Read the model definition and answer for the solid it produces. Units are mm, in the model's axes. Round coordinates to 2 decimals unless told otherwise and drop trailing zeros. Write each loop counter-clockwise with the first axis right and the second up, starting at its lowest first coordinate (ties: lowest second). Pieces come first, ordered by that corner, then holes. Notation, with made-up numbers: (62, 14) - (100, 14) arc R30 ccw to (100, 42) - close; hole circle Ø7 at (44, -29). An arc over 180 degrees is marked (long way). Use one line per item in the form item = value. Start each with the question number.
1) Consider line 1 along Z through (x, y) = (90, 3.65); line 2 along X through (y, z) = (4.3, -92); line 3 along X through (y, z) = (-2, 103). Determine where each line is inside the solid, lowest interval first. Write a range as from..to.
2) The part is cut by section C-C, the plane x = -90. Give the vertices of the cut face in (y, z).
3) This flat-tipped pin is pushed along its axis until it touches: pin 1 (3.5 mm diameter, centred on x = 88.5, z = 16, fed in from -Y). Where does it stop, or does it pass through?
4) The part is cut by section A-A, the plane z = 18. Give the vertices of the cut face in (x, y), plus the area to 3 significant figures.
5) The part is cut by section B-B, the plane x = 55. Give the vertices of the cut face in (y, z), plus the area to 3 significant figures.
from build123d import *

# Parameters (mm, degrees)
SKETCH_1_W                = 250
SKETCH_1_H                = 306
EXTRUDE_1_DEPTH           = 6
CHAMFER_1_SIZE            = 2
HOLE_WIZARD_M6_1_D        = 5
HOLE_WIZARD_M6_1_DEPTH    = 15
HOLE_WIZARD_M6_1_TIP      = 1.502151548
HOLE_WIZARD_M8_1_D        = 9
HOLE_WIZARD_1_D           = 6.6
HOLE_WIZARD_1_CBORE_D     = 11
HOLE_WIZARD_1_CBORE_DEPTH = 6.8
SKETCH_8_R                = 4
CUT_EXTRUDE_1_DEPTH       = 198.934332545
HOLE_WIZARD_M6_2_D        = 5
CHAMFER_2_SIZE            = 10


with BuildPart() as part:
    # 草图1 → 凸台-拉伸1 (new, symmetric)
    with BuildSketch(Plane(origin=(0, 0, 0), x_dir=(1, 0, 0), z_dir=(0, 1, 0))):
        Rectangle(SKETCH_1_W, SKETCH_1_H)
    extrude(amount=EXTRUDE_1_DEPTH, both=True)

    # 倒角1
    chamfer_1_edges = [part.edges().sort_by_distance(p)[0] for p in [
        (125, 0, 153),
        (-125, 0, 153),
    ]]
    chamfer(chamfer_1_edges, length=CHAMFER_1_SIZE)

    # M6 螺纹孔1
    with Locations(Plane(origin=(0, 0, -153), x_dir=(-1, 0, 0), z_dir=(0, 0, -1))):
        with Locations((-105, 0), (0, 0), (105, 0)):
            Hole(HOLE_WIZARD_M6_1_D / 2, depth=HOLE_WIZARD_M6_1_DEPTH)
            with Locations((0, 0, -(HOLE_WIZARD_M6_1_DEPTH + HOLE_WIZARD_M6_1_TIP / 2))):  # 118° drill point
                Cone(0, HOLE_WIZARD_M6_1_D / 2, HOLE_WIZARD_M6_1_TIP, mode=Mode.SUBTRACT)

    # M8 间隙孔1 (through all)
    with Locations(Plane(origin=(0, 6, 0), x_dir=(1, 0, 0), z_dir=(0, 1, 0))):
        with Locations((-105, -135.00000089), (-55, -135.00000089), (-105, 78.99999911), (-55, 78.99999911), (55, 78.99999911), (105, 78.99999911), (55, -135.00000089), (105, -135.00000089), (-35, -135.00000089), (35, -135.00000089), (-35, 78.99999911), (35, 78.99999911)):
            Hole(HOLE_WIZARD_M8_1_D / 2)

    # 打孔尺寸(%根据)内六角圆柱头螺钉的类型1 (through all)
    with Locations(Plane(origin=(0, -6, 0), x_dir=(-1, 0, 0), z_dir=(0, -1, 0))):
        with Locations((-90, -128), (-90, -18), (-90, 92), (90, 92), (90, -18), (90, -128)):
            CounterBoreHole(HOLE_WIZARD_1_D / 2, HOLE_WIZARD_1_CBORE_D / 2, HOLE_WIZARD_1_CBORE_DEPTH)

    # 草图8 → 切除-拉伸1 (cut, through all)
    with BuildSketch(Plane(origin=(0, 6, 0), x_dir=(1, 0, 0), z_dir=(0, 1, 0))):
        with Locations(Location((0, -135.00000089, 0), (0, 0, 270))):
            Circle(SKETCH_8_R)
        with BuildLine():
            Line((-4, 77.99999911), (-4, 79.99999911))
            ThreePointArc((-4, 79.99999911), (0, 83.99999911), (4, 79.99999911))
            Line((4, 79.99999911), (4, 77.99999911))
            ThreePointArc((4, 77.99999911), (0, 73.99999911), (-4, 77.99999911))
        make_face()
    extrude(amount=-CUT_EXTRUDE_1_DEPTH, mode=Mode.SUBTRACT)

    # M6 螺纹孔2 (through all)
    with Locations(Plane(origin=(0, 6, 0), x_dir=(1, 0, 0), z_dir=(0, 1, 0))):
        with Locations((25, -103), (-25, -103)):
            Hole(HOLE_WIZARD_M6_2_D / 2)

    # 倒角2
    chamfer_2_edges = [part.edges().sort_by_distance(p)[0] for p in [
        (-125, 0, -153),
        (125, 0, -153),
    ]]
    chamfer(chamfer_2_edges, length=CHAMFER_2_SIZE)


solid = part.part
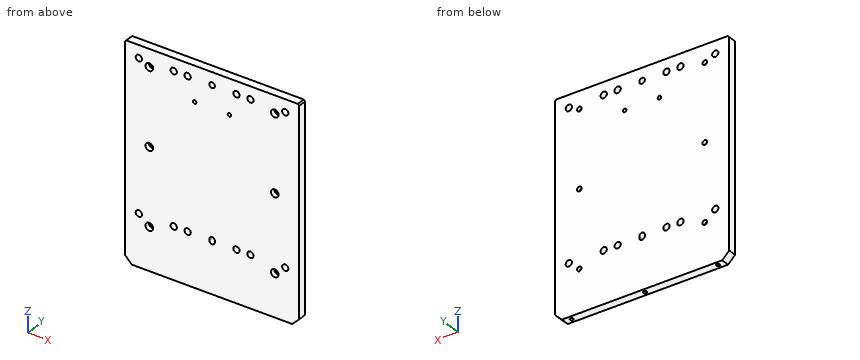
Geometry results:
q1.line_1 = -153..-95.3, -88.7..14.7, 21.3..124.7, 131.3..153
q1.line_2 = -125..-93.3, -86.7..86.7, 93.3..125
q1.line_3 = -125..-27.5, -22.5..22.5, 27.5..125
q2.outline = (-6, -153) - (6, -153) - (6, -95.3) - (0.8, -95.3) - (0.8, -97.5) - (-6, -97.5) - close; (-6, -86.5) - (0.8, -86.5) - (0.8, -88.7) - (6, -88.7) - (6, 14.7) - (0.8, 14.7) - (0.8, 12.5) - (-6, 12.5) - close; (-6, 23.5) - (0.8, 23.5) - (0.8, 21.3) - (6, 21.3) - (6, 124.7) - (0.8, 124.7) - (0.8, 122.5) - (-6, 122.5) - close; (-6, 133.5) - (0.8, 133.5) - (0.8, 131.3) - (6, 131.3) - (6, 153) - (-6, 153) - close
q3.pin_1 = 0.8
q4.outline = (-125, -6) - (-95.5, -6) - (-95.5, 0.8) - (-93.3, 0.8) - (-93.3, 6) - (-125, 6) - close; (-86.7, 0.8) - (-84.5, 0.8) - (-84.5, -6) - (84.5, -6) - (84.5, 0.8) - (86.7, 0.8) - (86.7, 6) - (-86.7, 6) - close; (93.3, 0.8) - (95.5, 0.8) - (95.5, -6) - (125, -6) - (125, 6) - (93.3, 6) - close
q4.area = 2,780 mm2
q5.outline = (-6, -153) - (6, -153) - (6, -83.5) - (-6, -83.5) - close; (-6, -74.5) - (6, -74.5) - (6, 130.5) - (-6, 130.5) - close; (-6, 139.5) - (6, 139.5) - (6, 153) - (-6, 153) - close
q5.area = 3,460 mm2
